```python
from build123d import *

# Parameters (mm, degrees)
EXTRUDE_1_DEPTH        = 5
HOLE_WIZARD_M5_1_D     = 4.2
HOLE_WIZARD_M5_1_DEPTH = 13
HOLE_WIZARD_M5_1_TIP   = 1.2618073
HOLE_WIZARD_M5_2_D     = 4.2
HOLE_WIZARD_M5_2_DEPTH = 14
HOLE_WIZARD_M5_2_TIP   = 1.2618073
HOLE_WIZARD_M3_1_D     = 2.5
HOLE_WIZARD_M3_1_DEPTH = 12.5
HOLE_WIZARD_M3_1_TIP   = 0.751075774


with BuildPart() as part:
    # 草图1 → 凸台-拉伸1 (new, symmetric)
    with BuildSketch(Plane.XY):
        Polygon((-68, 0), (-68, 15), (-28, 15), (-15, 50), (-15, 100), (0, 100), (0, 0), align=None)
    extrude(amount=EXTRUDE_1_DEPTH, both=True)

    # M5 螺纹孔1
    with Locations(Plane(origin=(0, 0, 0), x_dir=(-1, 0, 0), z_dir=(0, -1, 0))):
        with Locations((49, 0), (19, 0)):
            Hole(HOLE_WIZARD_M5_1_D / 2, depth=HOLE_WIZARD_M5_1_DEPTH)
            with Locations((0, 0, -(HOLE_WIZARD_M5_1_DEPTH + HOLE_WIZARD_M5_1_TIP / 2))):  # 118° drill point
                Cone(0, HOLE_WIZARD_M5_1_D / 2, HOLE_WIZARD_M5_1_TIP, mode=Mode.SUBTRACT)

    # M5 螺纹孔2
    with Locations(Plane(origin=(0, 0, 0), x_dir=(0, 0, -1), z_dir=(1, 0, 0))):
        with Locations((0, 30), (0, 90)):
            Hole(HOLE_WIZARD_M5_2_D / 2, depth=HOLE_WIZARD_M5_2_DEPTH)
            with Locations((0, 0, -(HOLE_WIZARD_M5_2_DEPTH + HOLE_WIZARD_M5_2_TIP / 2))):  # 118° drill point
                Cone(0, HOLE_WIZARD_M5_2_D / 2, HOLE_WIZARD_M5_2_TIP, mode=Mode.SUBTRACT)

    # M3 螺纹孔1
    with Locations(Plane(origin=(0, 15, 0), x_dir=(1, 0, 0), z_dir=(0, 1, 0))):
        with Locations((-58, 0), (-38, 0)):
            Hole(HOLE_WIZARD_M3_1_D / 2, depth=HOLE_WIZARD_M3_1_DEPTH)
            with Locations((0, 0, -(HOLE_WIZARD_M3_1_DEPTH + HOLE_WIZARD_M3_1_TIP / 2))):  # 118° drill point
                Cone(0, HOLE_WIZARD_M3_1_D / 2, HOLE_WIZARD_M3_1_TIP, mode=Mode.SUBTRACT)


solid = part.part
```
Build history of the part. All positions in model axes, mm. A direction names the side the tool comes from. Round coordinates to 2 decimals unless told otherwise and drop trailing zeros. Write each loop counter-clockwise with the first axis right and the second up, starting at its lowest first coordinate (ties: lowest second). Pieces come first, ordered by that corner, then holes. Notation, with made-up numbers: (-17, 34) -> (41, 34) arc R17 cw to (41, 50) -> close; hole circle Ø11 at (39, -35.5). An arc over 180 degrees is marked (long way). Put each result on its own line as item: value.
Item 1: Tool access for faces 1 (the face through (-36.75, 8.66, -0.05)), 2 (the face through (-16.997, 6.591, -0.631)), 3 (the face through (-48, 15, 0)): list every direction of +Z, -Z, +X, -X, +Y, -Y with a clear straight run to the whole face (end or side of a thin tool).
Here are the results:
face 1: +Y
face 2: -Y
face 3: +Z, -Z, -X, +Y
Item 2: Wall check: probe 1 along Y at (x, z) = (-6, 0); probe 2 along Z at (x, y) = (-49, 5); probe 3 along Z at (x, y) = (-58, 7.5). Give the ranges that are in metal, low to high. Write a range as from..to.
Here are the results:
probe 1: y = 0..27.9, 32.1..87.9, 92.1..100
probe 2: z = -5..-2.1, 2.1..5
probe 3: z = -5..-1.25, 1.25..5
Item 3: Slice it at C-C, the plane y = 67. Give the cut face in (x, z).
Here are the results:
outline: (-15, -5) -> (0, -5) -> (0, 5) -> (-15, 5) -> close
Item 4: Slice it at A-A, the plane z = 3.75. Give the cut face in (x, y).
Here are the results:
outline: (-68, 0) -> (0, 0) -> (0, 100) -> (-15, 100) -> (-15, 50) -> (-28, 15) -> (-68, 15) -> close
Item 5: Slice it at B-B, the plane x = -40.5. Give the cut face in (y, z), plus the area to 3 significant figures.
Here are the results:
outline: (0, -5) -> (15, -5) -> (15, 5) -> (0, 5) -> close
area: 150 mm^2
Item 6: Two-plate mould, pull along Y, no slides. Class faces 4 (the face through (-57.79, 1.88, -0.07)), 5 (the face through (-15.04, 30.31, -0.2)), 6 (the face through (-59.19, 8.66, -0.38)): pulls with the +Y half, pulls with the -Y half, needs draft (parallel to the pull), parting line crosses it, or undercut.
Here are the results:
face 4: pulls with the +Y half
face 5: undercut
face 6: needs draft
Item 7: Flat gauge pins, fed straight in: P1, Ø5, axis at y = 68.5, z = 2, coming from the -X side; P2, Ø5.5, axis at y = 30, z = 0, coming from the +X side; P3, Ø3.5, axis at x = -19, z = 0, coming from the -Y side; P4, Ø1, axis at y = 31.5, z = -2.5, coming from the -X side. Where does each tip first touch, or does it go through?
Here are the results:
P1: stops at x = -15
P2: stops at x = 0
P3: stops at y = 13.21
P4: stops at x = -22.06
